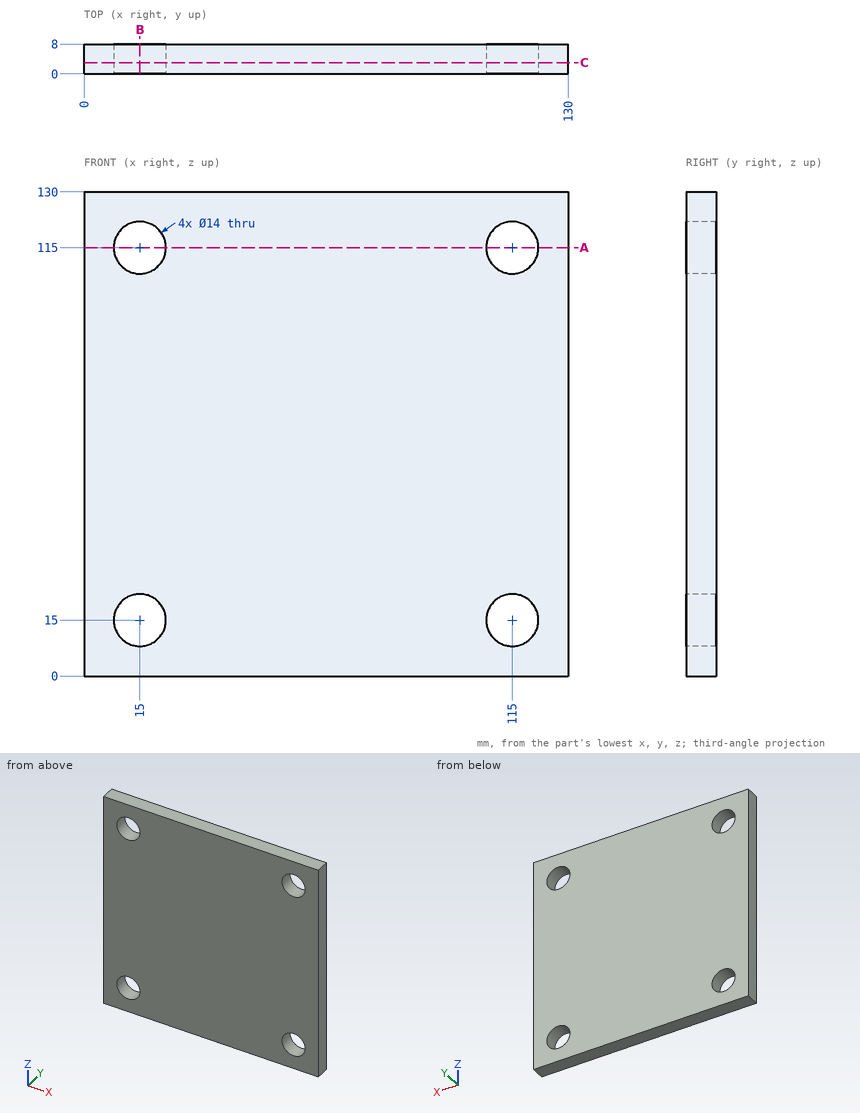
The figure shows three views and two pictorial views of one solid part (mm, origin at its lowest corner). Answer the questions. Give positions to 0.01 mm unless a question says otherwise; leave off trailing zeros. Loops run counter-clockwise (first coordinate to the right, second up) from the corner with the lowest first, then second, coordinate; pieces in that order, holes last. Notation, with made-up numbers: (14.5, 46.5) -> (56.5, 46.5) arc R17 ccw to (56.5, 59.5) -> close; hole circle Ø5 at (84, 64.25). An arc over 180 degrees is marked (long way). Put each result on its own line as item: value. Start each with the question number.
Item 1: The part is cut by section A-A (z = 115). Give the vertices of the cut face in (x, y).
Item 2: The part is cut by section C-C (y = 3). Give the vertices of the cut face in (x, z).
Item 3: The part is cut by section B-B (x = 15). Give the vertices of the cut face in (y, z).
Item 4: This flat-tipped pin is pushed along its axis until it touches: P1, Ø2, axis at y = 1.5, z = 109, coming from the -X side. Where does it stop, or does it pass through?
Item 5: Find the intervals of material crossed by L1, parallel to Z at x = 15, y = 5; L2, parallel to Z at x = 12, y = 1.75, in increasing order. Write a range as [from, to].
Answers below:
1. outline: (0, 0) -> (8, 0) -> (8, 8) -> (0, 8) -> close; (22, 0) -> (108, 0) -> (108, 8) -> (22, 8) -> close; (122, 0) -> (130, 0) -> (130, 8) -> (122, 8) -> close
2. outline: (0, 0) -> (130, 0) -> (130, 130) -> (0, 130) -> close; hole circle Ø14 at (15, 15); hole circle Ø14 at (15, 115); hole circle Ø14 at (115, 15); hole circle Ø14 at (115, 115)
3. outline: (0, 0) -> (8, 0) -> (8, 8) -> (0, 8) -> close; (0, 22) -> (8, 22) -> (8, 108) -> (0, 108) -> close; (0, 122) -> (8, 122) -> (8, 130) -> (0, 130) -> close
4. P1: x = 0
5. L1: [0, 8], [22, 108], [122, 130]
5. L2: [0, 8.68], [21.32, 108.68], [121.32, 130]
